Design review of the part shown in the three views and the two pictorial views. Dimensions are in mm from the part's minimum x, y and z. Give positions to 0.01 mm unless a question says otherwise; leave off trailing zeros. Loops run counter-clockwise (first coordinate to the right, second up) from the corner with the lowest first, then second, coordinate; pieces in that order, holes last. Notation, with made-up numbers: (25.25, 53.5) - (37.25, 53.5) arc R10 cw to (37.25, 61.5) - close; hole circle Ø3 at (51.5, 68). An arc over 180 degrees is marked (long way). Put each result on its own line as item: value. Start each with the question number.
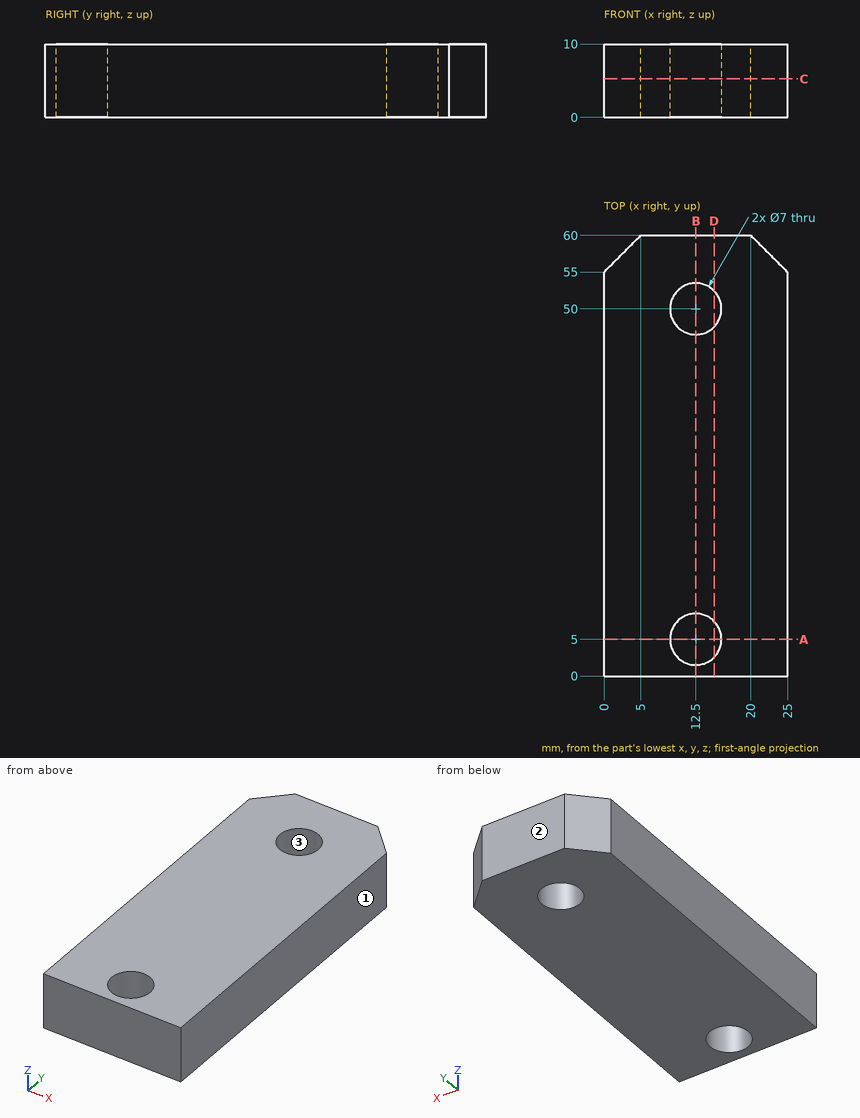
1) Wall thickness on probe 1 along Y at (x, z) = (12.5, 3.75); probe 2 along Y at (x, z) = (9.5, 8.75); probe 3 along X at (y, z) = (8, 7.25): over which ranges is each line inside the solid? List them lowest first.
2) Take a section at B-B on x = 12.5. State the section outline as (y, z) points, and give its area (3 significant figures).
3) Take a section at D-D on x = 15. State the section outline as (y, z) points, and give its area (3 significant figures).
4) Take a section at C-C on z = 5.25. State the section outline as (x, y) points.
5) Take a section at A-A on y = 5. State the section outline as (x, z) points.
6) Insertion check: P1, Ø6, axis at y = 20.5, z = 1.5, coming from the -X side. The pin has a flat end and moves straight along its axis. Give the tip position at first contact, or say it passes through.
7) Mouldability with a two-part tool opening along Y and no side actions: class the marked faces 1, 2 and 3 as released by +Y, released by -Y, zero draft, split by the parting line, or undercut.
Answers follow:
1. probe 1: 0 to 1.5, 8.5 to 46.5, 53.5 to 60
1. probe 2: 0 to 3.2, 6.8 to 48.2, 51.8 to 60
1. probe 3: 0 to 10.7, 14.3 to 25
2. outline: (0, 0) - (1.5, 0) - (1.5, 10) - (0, 10) - close; (8.5, 0) - (46.5, 0) - (46.5, 10) - (8.5, 10) - close; (53.5, 0) - (60, 0) - (60, 10) - (53.5, 10) - close
2. area: 460 mm2
3. outline: (0, 0) - (2.55, 0) - (2.55, 10) - (0, 10) - close; (7.45, 0) - (47.55, 0) - (47.55, 10) - (7.45, 10) - close; (52.45, 0) - (60, 0) - (60, 10) - (52.45, 10) - close
3. area: 502 mm2
4. outline: (0, 0) - (25, 0) - (25, 55) - (20, 60) - (5, 60) - (0, 55) - close; hole circle Ø7 at (12.5, 5); hole circle Ø7 at (12.5, 50)
5. outline: (0, 0) - (9, 0) - (9, 10) - (0, 10) - close; (16, 0) - (25, 0) - (25, 10) - (16, 10) - close
6. P1: x = 0
7. face 1: zero draft
7. face 2: released by +Y
7. face 3: undercut
